Verification items for this drawing (mm, ordinates from the low corner). A direction names the side the tool comes from. Round coordinates to 2 decimals unless told otherwise and drop trailing zeros. Loops run counter-clockwise (first coordinate to the right, second up) from the corner with the lowest first, then second, coordinate; pieces in that order, holes last. Notation, with made-up numbers: M -26.5,38 L 23.5,38 A25 ccw 23.5,61 Z; hole C -25,-27 d4. An arc over 180 degrees is marked long. Write item = value, one per line. Start each with the question number.
(1) Cross-section at B-B on z = 4.5. Record the boundary of the cut face in (x, y), plus the area to 3 significant figures.
(2) Mould release check, pull along X, two halves, no side actions. Record for the marked faces 3 and 4: pulls with the +X half, pulls with the -X half, needs draft (parallel to the pull), parting line crosses it, or undercut.
(3) Go/stop test with flat-tipped pins: P1, Ø10, axis at x = 41, y = 42, coming from the +Z side; P2, Ø6, axis at x = 90, z = 6.5, coming from the +Y side. Record where each tip stops, or that it passes through.
(4) Scan lines: L1, parallel to X at y = 83, z = 3.5; L2, parallel to Y at x = 17, z = 9.5; L3, parallel to X at y = 72.5, z = 6.75. Record each from-to range of solid material in increasing order. Write a range as from..to.
(5) Cross-section at A-A on y = 34. Record the boundary of the cut face in (x, z).
(6) Cross-section at C-C on x = 17. Record the boundary of the cut face in (y, z), plus the area to 3 significant figures.
(7) Set-up check for the marked faces 1 and 2: record each of +Z, -Z, +X, -X, +Y, -Y from which the full face is reachable in a straight line by a thin tool's end or side.
(8) Cross-section at D-D on y = 75. Record the boundary of the cut face in (x, z).
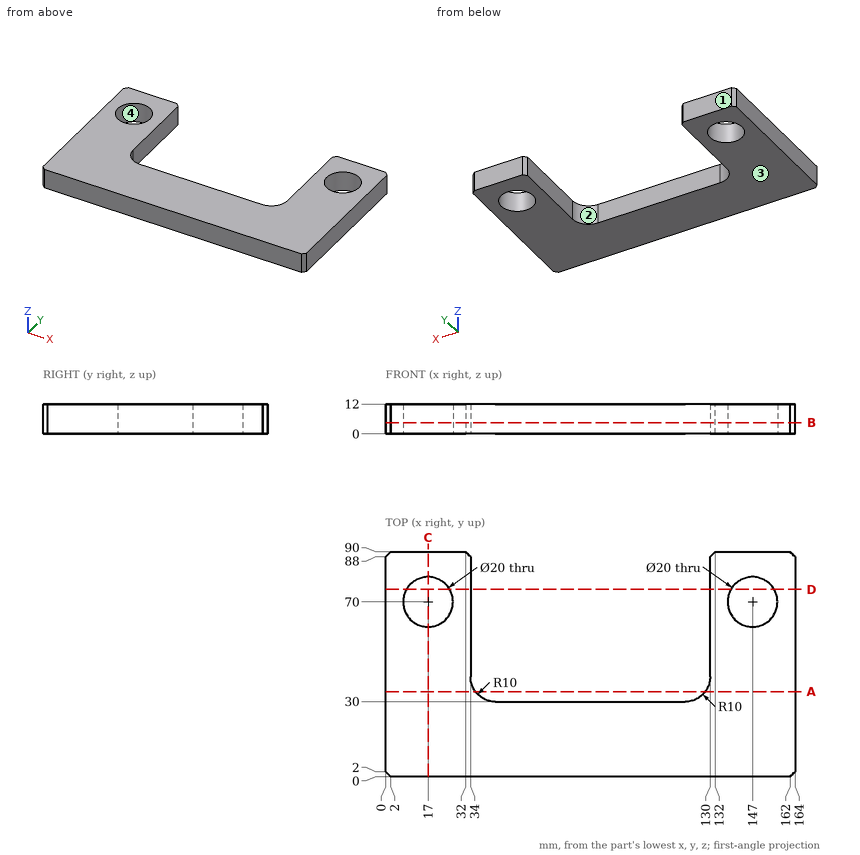
Result:
q1.outline = M 0,2 L 2,0 L 162,0 L 164,2 L 164,88 L 162,90 L 132,90 L 130,88 L 130,40 A10 cw 120,30 L 44,30 A10 cw 34,40 L 34,88 L 32,90 L 2,90 L 0,88 Z; hole C 17,70 d20; hole C 147,70 d20
q1.area = 8,400 mm^2
q2.face_3 = needs draft
q2.face_4 = undercut
q3.P1 = through
q3.P2 = 30
q4.L1 = 0..34, 130..164
q4.L2 = 0..60, 80..90
q4.L3 = 0..7.32, 26.68..34, 130..137.32, 156.68..164
q5.outline = M 0,0 L 36,0 L 36,12 L 0,12 Z; M 128,0 L 164,0 L 164,12 L 128,12 Z
q6.outline = M 0,0 L 60,0 L 60,12 L 0,12 Z; M 80,0 L 90,0 L 90,12 L 80,12 Z
q6.area = 840 mm^2
q7.face_1 = +Z, -Z, +X, -X, +Y
q7.face_2 = +Z, -Z, +Y
q8.outline = M 0,0 L 8.34,0 L 8.34,12 L 0,12 Z; M 25.66,0 L 34,0 L 34,12 L 25.66,12 Z; M 130,0 L 138.34,0 L 138.34,12 L 130,12 Z; M 155.66,0 L 164,0 L 164,12 L 155.66,12 Z
